from build123d import *

# Parameters (mm, degrees)
SKETCH_1_W          = 63
SKETCH_1_H          = 130.5
EXTRUDE_1_DEPTH     = 1.5
EXTRUDE_START       = 1.5
SKETCH_2_W          = 123
SKETCH_2_H          = 88
EXTRUDE_2_DEPTH     = 93
SKETCH_3_R          = 44
EXTRUDE_3_DEPTH     = 115.5
SKETCH_5_W          = 63
SKETCH_5_H          = 88
EXTRUDE_4_DEPTH     = 3
SKETCH_6_R          = 6
CUT_EXTRUDE_2_DEPTH = 238.323750392
SKETCH_4_R          = 12.5
CUT_EXTRUDE_1_DEPTH = 238.323750392
FILLET_1_R          = 5


with BuildPart() as part:
    # Sketch 1 → Extrude 1 (new body)
    with BuildSketch(Plane(origin=(0, 0, 0), x_dir=(1, 0, 0), z_dir=(0, 1, 0))):
        Rectangle(SKETCH_1_W, SKETCH_1_H)
    extrude(amount=EXTRUDE_1_DEPTH)



with BuildPart() as body_2:
    # Sketch 2 → Extrude 2 (new body)
    with BuildSketch(Plane.XZ.offset(EXTRUDE_START)):
        with Locations((30, 0)):
            Rectangle(SKETCH_2_W, SKETCH_2_H)
    extrude(amount=EXTRUDE_2_DEPTH)

    # Sketch 3 → Extrude 3 (add)
    with BuildSketch(Plane(origin=(91.5, 0, 0), x_dir=(0, 0, -1), z_dir=(1, 0, 0))):
        with Locations((0, -48)):
            Circle(SKETCH_3_R)
    extrude(amount=EXTRUDE_3_DEPTH)


with BuildPart() as part_1:
    add(part.part)

    add(body_2.part)  # Extrude 4 merges body 2
    # Sketch 5 → Extrude 4 (add)
    with BuildSketch(Plane.XZ):
        Rectangle(SKETCH_5_W, SKETCH_5_H)
    extrude(amount=EXTRUDE_4_DEPTH)

    # Sketch 6 → Cut-Extrude 2 (cut, through all)
    with BuildSketch(Plane(origin=(0, 1.5, 0), x_dir=(1, 0, 0), z_dir=(0, 1, 0))):
        with Locations(Location((-20.25, 55.25, 0), (0, 0, 270))):
            Circle(SKETCH_6_R)
        with Locations(Location((20.25, 55.25, 0), (0, 0, 270))):
            Circle(SKETCH_6_R)
        with Locations(Location((-20.25, -55.25, 0), (0, 0, 270))):
            Circle(SKETCH_6_R)
        with Locations(Location((20.25, -55.25, 0), (0, 0, 270))):
            Circle(SKETCH_6_R)
    extrude(amount=-CUT_EXTRUDE_2_DEPTH, mode=Mode.SUBTRACT)

    # Sketch 4 → Cut-Extrude 1 (cut, through all)
    with BuildSketch(Plane(origin=(0, 1.5, 0), x_dir=(1, 0, 0), z_dir=(0, 1, 0))):
        with Locations(Location((0, 0, 0), (0, 0, 270))):
            Circle(SKETCH_4_R)
    extrude(amount=-CUT_EXTRUDE_1_DEPTH, mode=Mode.SUBTRACT)

    # Fillet 1
    fillet_1_edges = [part_1.edges().sort_by_distance(p)[0] for p in [
        (207, -48, 44),
    ]]
    fillet(fillet_1_edges, radius=FILLET_1_R)


solid = part_1.part
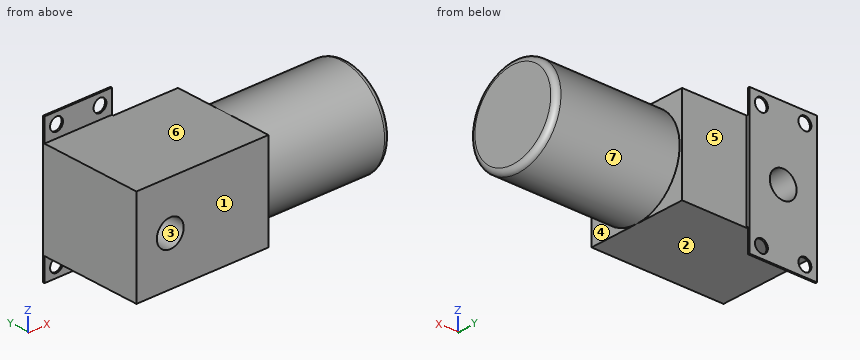
Can you work these out from the model? Positions are in its coordinate system, mm. Face numbers are marked on the shaded views. A direction names the side the tool comes from. Round coordinates to 2 decimals unless told otherwise and drop trailing zeros. Write each loop counter-clockwise with the first axis right and the second up, starting at its lowest first coordinate (ties: lowest second). Pieces come first, ordered by that corner, then holes. Notation, with made-up numbers: M 7,41.5 L 38,41.5 A23 ccw 38,71.5 Z; hole C 33.5,35.25 d9. An arc over 180 degrees is marked long. Use a Markdown table: item, result.
Item 1: I want a section at B-B (z = 55.25). List the corners of the cut face in (x, y) for me.
Found:
| item | result |
|---|---|
| outline | M -31.5,0 L -26.25,0 L -26.25,1.5 L -31.5,1.5 Z; M -14.25,0 L 14.25,0 L 14.25,1.5 L -14.25,1.5 Z; M 26.25,0 L 31.5,0 L 31.5,1.5 L 26.25,1.5 Z |
Item 2: For pin 1 Ø14 at (x, z) = (-20.25, 55.25) entering from -Y; pin 2 Ø2 at (x, y) = (19, -21) entering from -Z; pin 3 Ø6 at (x, z) = (172, -43) entering from +Y, each with a flat end and sliding along its axis, tell me the tip position at first contact or that it passes through.
Found:
| item | result |
|---|---|
| pin 1 | stops at y = 0 |
| pin 2 | stops at z = -44 |
| pin 3 | stops at y = -29.67 |
Item 3: Which directions (+Z, -Z, +X, -X, +Y, -Y) give clear straight access to the entire face, cutting with the end or side of a thin tool? Please do the marked faces 4, 5, 6 and 7.
Found:
| item | result |
|---|---|
| face 4 | +X, -Y |
| face 5 | +Z, -Z, +X, +Y |
| face 6 | +Z, +X, -X, -Y |
| face 7 | +X |
Item 4: I want a section at A-A (x = 0). List the corners of the cut face in (y, z) for me, and give its area (3 significant figures).
Found:
| item | result |
|---|---|
| outline | M -94.5,-44 L 0,-44 L 0,-65.25 L 1.5,-65.25 L 1.5,-12.5 L -94.5,-12.5 Z; M -94.5,12.5 L 1.5,12.5 L 1.5,65.25 L 0,65.25 L 0,44 L -94.5,44 Z |
| area | 6,110 mm2 |
Item 5: We'd pull the mould along Z, two halves only. Please class the marked faces 1, 2 and 3: released by +Z, released by -Z, zero draft, split by the parting line, or undercut.
Found:
| item | result |
|---|---|
| face 1 | zero draft |
| face 2 | released by -Z |
| face 3 | undercut |
Item 6: I want a section at C-C (z = 0). List the corners of the cut face in (x, y) for me.
Found:
| item | result |
|---|---|
| outline | M -31.5,-94.5 L -12.5,-94.5 L -12.5,1.5 L -31.5,1.5 Z; M 12.5,-94.5 L 91.5,-94.5 L 91.5,-92 L 202,-92 A5 ccw 207,-87 L 207,-9 A5 ccw 202,-4 L 91.5,-4 L 91.5,-1.5 L 31.5,-1.5 L 31.5,1.5 L 12.5,1.5 Z |
Item 7: I want a section at D-D (x = 149). List the corners of the cut face in (y, z) for me.
Found:
| item | result |
|---|---|
| outline | C -48,0 d88 |
Item 8: If I drill on line 1 along Z through (x, y) = (-20, 1); line 2 along X through (y, z) = (0.4, -55.25); line 3 along Y through (x, z) = (45, -26), over which ranges is the centre line in solid material (lowest first)? Write a range as [from, to].
Found:
| item | result |
|---|---|
| line 1 | z = [-65.25, -61.24], [-49.26, 49.26], [61.24, 65.25] |
| line 2 | x = [-31.5, -26.25], [-14.25, 14.25], [26.25, 31.5] |
| line 3 | y = [-94.5, -1.5] |
